```python
from build123d import *

# Parameters (mm, degrees)
BASE_PLATE_SKETCH_W        = 120
BASE_PLATE_SKETCH_H        = 80
BASE_PLATE_120X80X15_DEPTH = 15
BORE_30_SKETCH_R           = 15
BORE_30_DEPTH              = 15
HUB_BOSS_SKETCH_R          = 40
HUB_BOSS_SKETCH_R_2        = 30
HUB_BOSS_DEPTH             = 20
HUB_INNER_STEP_SKETCH_R    = 30
HUB_INNER_STEP_SKETCH_R_2  = 15
HUB_INNER_STEP_DEPTH       = 5
LUG_A_SKETCH_R             = 16
LUG_A_DEPTH                = 20
LUG_START                  = -20
LUG_B_SKETCH_R             = 16
LUG_B_DEPTH                = 20


with BuildPart() as part:
    # Base Plate Sketch → Base Plate 120x80x15 (new body)
    with BuildSketch(Plane.XY):
        Rectangle(BASE_PLATE_SKETCH_W, BASE_PLATE_SKETCH_H)
    extrude(amount=BASE_PLATE_120X80X15_DEPTH)

    # Bore Ø30 Sketch → Bore Ø30 (cut)
    with BuildSketch(Plane(origin=(0, 0, 0), x_dir=(-1, 0, 0), z_dir=(0, 0, -1))):
        Circle(BORE_30_SKETCH_R)
    extrude(amount=-BORE_30_DEPTH, mode=Mode.SUBTRACT)

    # Hub Boss Sketch → Hub Boss (add)
    with BuildSketch(Plane.XY.offset(15)):
        with Locations(Location((0, 0, 0), (0, 0, 270))):
            Circle(HUB_BOSS_SKETCH_R)
        Circle(HUB_BOSS_SKETCH_R_2, mode=Mode.SUBTRACT)
    extrude(amount=HUB_BOSS_DEPTH)

    # Hub Inner Step Sketch → Hub Inner Step (add)
    with BuildSketch(Plane.XY.offset(15)):
        Circle(HUB_INNER_STEP_SKETCH_R)
        with Locations(Location((0, 0, 0), (0, 0, 180))):
            Circle(HUB_INNER_STEP_SKETCH_R_2, mode=Mode.SUBTRACT)
    extrude(amount=HUB_INNER_STEP_DEPTH)

    # Lug A Sketch → Lug A (add)
    with BuildSketch(Plane(origin=(60, 0, 0), x_dir=(0, 0, -1), z_dir=(1, 0, 0))):
        with BuildLine():
            Line((0, 40), (40, 40))
            ThreePointArc((40, 40), (80, 0), (40, -40))
            Line((40, -40), (0, -40))
            Line((0, -40), (0, 40))
        make_face()
        with Locations((40, 0)):
            Circle(LUG_A_SKETCH_R, mode=Mode.SUBTRACT)
    extrude(amount=-LUG_A_DEPTH)

    # Lug B Sketch → Lug B (add)
    with BuildSketch(Plane.ZY.offset(60).offset(LUG_START)):
        with BuildLine():
            Line((-40, 40), (15, 40))
            Line((15, 40), (15, -40))
            Line((15, -40), (-40, -40))
            ThreePointArc((-40, -40), (-80, 0), (-40, 40))
        make_face()
        with Locations(Location((-40, 0, 0), (0, 0, 180))):
            Circle(LUG_B_SKETCH_R, mode=Mode.SUBTRACT)
    extrude(amount=LUG_B_DEPTH)


solid = part.part
```
Could you check a few things on this model? Use its own coordinates, in mm. A direction names the side the tool comes from. Give positions to 0.01 mm unless a question says otherwise; leave off trailing zeros. Order: outer loops, then holes, each group sorted by start corner. A loop starts at its lowest first (then second) coordinate and runs counter-clockwise, first axis right, second up.
Q1. Suppose I cut it at A-A, the plane x = 43. Write out the boundary of the cut face in (y, z), and give its area (3 significant figures).
Q2. We'd pull the mould along Z, two halves only. Please class faces 1 (the cylindrical face through (50.14, 0.703, -24.015)), 2 (the cylindrical face through (50.14, 0.88, -79.99)), 3 (the flat face through (43, 1, 15)): +Z half, -Z half, draft (parallel to the pull), parting line (faces both ways), or undercut.
Q3. If I drill on line 1 along X through (y, z) = (3.5, -59); line 2 along Y through (x, z) = (0, 18.5); line 3 along Y through (x, z) = (55, -40), over which ranges is the centre line in solid material (lowest first)?
Q4. Suppose I cut it at C-C, the plane x = -3.5. Write out the boundary of the cut face in (y, z), and give its area (3 significant figures).
Q5. I'm going to push flat-ended pins straight in: P1, Ø6, axis at x = -38, y = 13.5, coming from the +Z side; P2, Ø1.5, axis at x = -41.5, z = -64, coming from the -Y side; P3, Ø19, axis at y = 0, z = -40, coming from the +X side; P4, Ø5, axis at x = -9, y = -17.5, coming from the -Z side. Where does each tip first touch, or does it pass through?
Q6. For faces 4 (the cylindrical face through (-39.05, 8.67, 24.86)), 5 (the flat face through (-44, 1, 15)), 6 (the flat face through (40, 1, -23)), which set-ups out of +Z, -Z, +X, -X, +Y, -Y let a thin tool reach every point of the face, with its end or its side?
Q7. Suppose I cut it at B-B, the plane y = 0. Write out the boundary of the cut face in (x, z).
Q8. Suppose I cut it at D-D, the plane z = 25. Write out the boundary of the cut face in (x, y).
Solution:
1. outline: (-40, -40) arc R40 ccw to (40, -40) - (40, 15) - (-40, 15) - close; hole circle Ø32 at (0, -40)
1. area: 6,110 mm2
2. face 1: undercut
2. face 2: -Z half
2. face 3: +Z half
3. line 1: x = -60 to -40, 40 to 60
3. line 2: y = -40 to -15, 15 to 40
3. line 3: y = -40 to -16, 16 to 40
4. outline: (-40, 0) - (-14.59, 0) - (-14.59, 20) - (-29.8, 20) - (-29.8, 35) - (-39.85, 35) - (-39.85, 15) - (-40, 15) - close; (14.59, 0) - (40, 0) - (40, 15) - (39.85, 15) - (39.85, 35) - (29.8, 35) - (29.8, 20) - (14.59, 20) - close
4. area: 1,320 mm2
5. P1: stops at z = 35
5. P2: stops at y = -32.55
5. P3: passes through
5. P4: stops at z = 0
6. face 4: +Z
6. face 5: +Z, -X
6. face 6: -Z, +Y, -Y
7. outline: (-60, -80) - (-40, -80) - (-40, -56) - (-60, -56) - close; (-60, -24) - (-40, -24) - (-40, 0) - (-15, 0) - (-15, 20) - (-30, 20) - (-30, 35) - (-40, 35) - (-40, 15) - (-60, 15) - close; (15, 0) - (40, 0) - (40, -24) - (60, -24) - (60, 15) - (40, 15) - (40, 35) - (30, 35) - (30, 20) - (15, 20) - close; (40, -80) - (60, -80) - (60, -56) - (40, -56) - close
8. outline: circle Ø80 at (0, 0); hole circle Ø60 at (0, 0)
